```python
from build123d import *

# Parameters (mm, degrees)
BLOCK_PROFILE_SKETCH_W  = 64
BLOCK_PROFILE_SKETCH_H  = 64
BLOCK_BODY_DEPTH        = 70
CROSS_HOLE_A_SKETCH_R   = 17.5
CROSS_HOLE_A_DEPTH      = 101.09995005
CROSS_HOLE_B_SKETCH_R   = 17.5
CROSS_HOLE_B_DEPTH      = 101.09995005
EDGE_CHAMFERS_5X45_SIZE = 5


with BuildPart() as part:
    # Block Profile Sketch → Block Body (new body)
    with BuildSketch(Plane.XY):
        Rectangle(BLOCK_PROFILE_SKETCH_W, BLOCK_PROFILE_SKETCH_H)
    extrude(amount=BLOCK_BODY_DEPTH)

    # Cross Hole A Sketch → Cross Hole A (cut, through all)
    with BuildSketch(Plane(origin=(0, 32, 0), x_dir=(1, 0, 0), z_dir=(0, 1, 0))):
        with Locations(Location((0, -35, 0), (0, 0, 180))):
            Circle(CROSS_HOLE_A_SKETCH_R)
    extrude(amount=-CROSS_HOLE_A_DEPTH, mode=Mode.SUBTRACT)

    # Cross Hole B Sketch → Cross Hole B (cut, through all)
    with BuildSketch(Plane(origin=(32, 0, 0), x_dir=(0, 0, -1), z_dir=(1, 0, 0))):
        with Locations(Location((-35, 0, 0), (0, 0, 90))):
            Circle(CROSS_HOLE_B_SKETCH_R)
    extrude(amount=-CROSS_HOLE_B_DEPTH, mode=Mode.SUBTRACT)

    # Edge Chamfers 5x45°
    edge_chamfers_5x45_edges = [part.edges().sort_by_distance(p)[0] for p in [
        (32, 0, 70),
        (0, 32, 70),
        (-32, 0, 70),
        (0, 32, 0),
        (32, 0, 0),
        (-32, 0, 0),
        (-32, 32, 35),
        (32, 32, 35),
        (32, -32, 35),
        (-32, -32, 35),
        (0, -32, 70),
    ]]
    chamfer(edge_chamfers_5x45_edges, length=EDGE_CHAMFERS_5X45_SIZE)


solid = part.part
```
Work out the finished part from the listing and answer in its coordinate system (mm). Give positions to 0.01 mm unless a question says otherwise; leave off trailing zeros. Order: outer loops, then holes, each group sorted by start corner. A loop starts at its lowest first (then second) coordinate and runs counter-clockwise, first axis right, second up. Notation, with made-up numbers: M 22,66.5 L 61,66.5 A18 ccw 61,70.5 Z; hole C 75,77.25 d1. An arc over 180 degrees is marked long. Return JSON: item names as keys, results as strings.
1) Section C-C, the plane x = 7 is taken. Write down the section's boundary in (y, z).
Resolved:
{"outline": "M -32,0 L 27,0 L 32,5 L 32,18.96 L 7,18.96 A17.5 cw -7,18.96 L -32,18.96 Z; M -32,51.04 L -7,51.04 A17.5 cw 7,51.04 L 32,51.04 L 32,65 L 27,70 L -27,70 L -32,65 Z"}
2) Section D-D, the plane y = 5.5 is taken. Write down the section's boundary in (x, z), plus the area to 3 significant figures.
Resolved:
{"outline": "M -32,5 L -27,0 L 27,0 L 32,5 L 32,18.39 L 5.5,18.39 A17.5 cw -5.5,18.39 L -32,18.39 Z; M -32,51.61 L -5.5,51.61 A17.5 cw 5.5,51.61 L 32,51.61 L 32,65 L 27,70 L -27,70 L -32,65 Z", "area": "2,290 mm^2"}
3) Straight lines are drawn through the part: line 1 along Z through (x, y) = (0, 25); line 2 along Y through (x, z) = (20.5, 35). For each, find the intervals that lie inside material, in ascending order. Write a range as [from, to].
Resolved:
{"line 1": "[0, 17.5], [52.5, 70]", "line 2": "[-32, -17.5], [17.5, 32]"}
4) Section B-B, the plane z = 48.5 is taken. Write down the section's boundary in (x, y).
Resolved:
{"outline": "M -32,-27 L -27,-32 L -11.14,-32 L -11.14,-11.14 L -32,-11.14 Z; M -32,11.14 L -11.14,11.14 L -11.14,32 L -27,32 L -32,27 Z; M 11.14,-32 L 27,-32 L 32,-27 L 32,-11.14 L 11.14,-11.14 Z; M 11.14,11.14 L 32,11.14 L 32,27 L 27,32 L 11.14,32 Z"}
5) For a pull along X with two mould halves and no side action, classify faces 1 (the flat face through (28.9, 28.5, 3.4)), 2 (the cylindrical face through (-8.075, 19.78, 19.474)), 3 (the flat face through (0, 30, 67)), 4 (the flat face through (-29, 0, 68)) as +X half, -X half, draft (parallel to the pull), parting line (faces both ways), or undercut.
Resolved:
{"face 1": "+X half", "face 2": "undercut", "face 3": "draft", "face 4": "-X half"}
6) Section A-A, the plane y = -26 is taken. Write down the section's boundary in (x, z).
Resolved:
{"outline": "M -32,5 L -27,0 L 27,0 L 32,5 L 32,65 L 27,70 L -27,70 L -32,65 Z; hole C 0,35 d35"}
